Read the model definition and answer for the solid it produces. Units are mm, in the model's axes. Give positions to 0.01 mm unless a question says otherwise; leave off trailing zeros. Write each loop counter-clockwise with the first axis right and the second up, starting at its lowest first coordinate (ties: lowest second). Pieces come first, ordered by that corner, then holes. Notation, with made-up numbers: (56, 68) - (82, 68) arc R34 cw to (82, 104) - close; hole circle Ø5 at (67.25, -39.75). An arc over 180 degrees is marked (long way). Answer as CSV lines item,"result".
```python
from build123d import *

# Parameters (mm, degrees)
SKETCH1_W           = 40
SKETCH1_H           = 40
SKETCH1_W_2         = 36
SKETCH1_H_2         = 36
BOSS_EXTRUDE1_DEPTH = 1082
FILLET1_R           = 2
FILLET2_R           = 4


with BuildPart() as part:
    # Sketch1 → Boss-Extrude1 (new body)
    with BuildSketch(Plane.XY):
        Rectangle(SKETCH1_W, SKETCH1_H)
        Rectangle(SKETCH1_W_2, SKETCH1_H_2, mode=Mode.SUBTRACT)
    extrude(amount=BOSS_EXTRUDE1_DEPTH)

    # Fillet1
    fillet1_edges = [part.edges().sort_by_distance(p)[0] for p in [
        (18, -18, 541),
        (18, 18, 541),
        (-18, 18, 541),
        (-18, -18, 541),
    ]]
    fillet(fillet1_edges, radius=FILLET1_R)

    # Fillet2
    fillet2_edges = [part.edges().sort_by_distance(p)[0] for p in [
        (20, -20, 541),
        (-20, -20, 541),
        (-20, 20, 541),
        (20, 20, 541),
    ]]
    fillet(fillet2_edges, radius=FILLET2_R)


solid = part.part
```
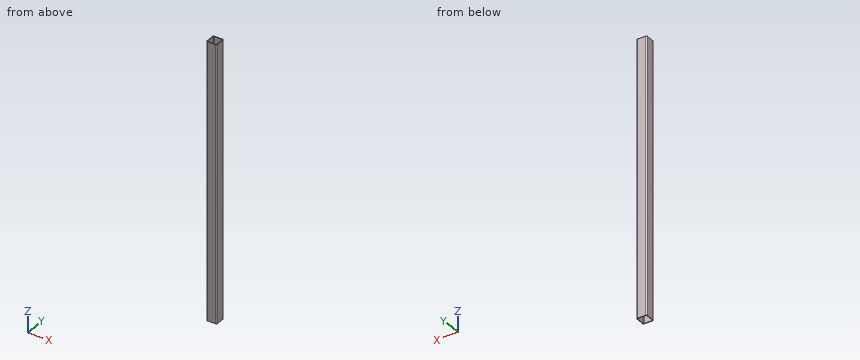
(1) A cutting plane is placed at C-C (z = 270.5). Write down the section's boundary in (x, y), and give its area (3 significant figures).
Worked out:
outline,"(-20, -16) arc R4 ccw to (-16, -20) - (16, -20) arc R4 ccw to (20, -16) - (20, 16) arc R4 ccw to (16, 20) - (-16, 20) arc R4 ccw to (-20, 16) - close; hole (-18, -16) arc R2 ccw to (-16, -18) - (16, -18) arc R2 ccw to (18, -16) - (18, 16) arc R2 ccw to (16, 18) - (-16, 18) arc R2 ccw to (-18, 16) - close"
area,"294 mm^2"
(2) This flat-tipped pin is pushed along its axis until it touches: P1, Ø4, axis at x = -14.5, y = 5, coming from the +Z side. Where does it stop, or does it pass through?
Worked out:
P1,"passes through"
(3) A cutting plane is placed at A-A (y = 3.5). Write down the section's boundary in (x, z).
Worked out:
outline,"(-20, 0) - (-18, 0) - (-18, 1082) - (-20, 1082) - close; (18, 0) - (20, 0) - (20, 1082) - (18, 1082) - close"
(4) Find the intervals of material crossed by L1, parallel to Y at x = -12.5, z = 944, in increasing order.
Worked out:
L1,"y = -20 to -18, 18 to 20"
